Verification items for the finished model (mm, model axes). A direction names the side the tool comes from. Coordinates: 2 decimals unless noted, no trailing zeros. Order: outer loops, then holes, each group sorted by start corner. A loop starts at its lowest first (then second) coordinate and runs counter-clockwise, first axis right, second up. Notation, with made-up numbers: M 24,0.25 L 31,0.25 A27 ccw 31,25.25 Z; hole C -40,-28.75 d1. An arc over 180 degrees is marked long. Return JSON: item names as keys, results as strings. Group by question number.
1. Section check B-B, the plane z = -107. Record the cut outline in (x, y), plus the area to 3 significant figures.
2. Material ranges on line 1 along X through (y, z) = (258, 5); line 2 along Z through (x, y) = (-108, 240), recorded low to high.
3. Mould release check, pull along X, two halves, no side actions. Record for faces 1 (the flat face through (5, 143, -176.332)), 2 (the flat face through (9, 143, -171.332)), 3 (the flat face through (-143.106, 111, -22)), 4 (the flat face through (151.894, 143, 13)): +X half, -X half, draft (parallel to the pull), parting line (faces both ways), or undercut.
4. Section check C-C, the plane z = 100. Record the cut outline in (x, y), plus the area to 3 significant figures.
5. Section check D-D, the plane y = 256. Record the cut outline in (x, z), plus the area to 3 significant figures.
6. Set-up check for faces 5 (the flat face through (-138.106, 111, -23)), 6 (the flat face through (74.3, 290, -171.5)): record each of +Z, -Z, +X, -X, +Y, -Y from which the full face is reachable in a straight line by a thin tool's end or side.
7. Gauge pin test, flat ends, axial feed: pin 1 (2.5 mm diameter, centred on x = 154.39, y = 25, fed in from -Z); pin 2 (5 mm diameter, centred on x = -35.5, y = 87, fed in from +Z); pin 3 (1.2 mm diameter, centred on x = 154.39, z = 73.67, fed in from -Y). Record the tip position at first contact, or that the pin passes through.
8. Section check A-A, the plane z = 18. Record the cut outline in (x, y).
```python
from build123d import *

# Parameters (mm, degrees)
BOSS_EXTRUDE1_DEPTH         = 290
M2_5_TAPPED_HOLE1_D         = 2.05
M2_5_TAPPED_HOLE1_DEPTH     = 7.25
M2_5_TAPPED_HOLE1_TIP       = 0.615882135
CUT_EXTRUDE2_DEPTH          = 41
CUT_EXTRUDE3_DEPTH          = 56
M4_TAPPED_HOLE1_D           = 3.3
M4_TAPPED_HOLE1_CSINK_D     = 4.05
M4_TAPPED_HOLE1_CSINK_ANGLE = 90
M2_5_TAPPED_HOLE2_D         = 2.05
M2_5_TAPPED_HOLE2_DEPTH     = 7.25
M2_5_TAPPED_HOLE2_TIP       = 0.615882135


with BuildPart() as part:
    # Sketch1 → Boss-Extrude1 (new body)
    with BuildSketch(Plane(origin=(0, 0, 0), x_dir=(1, 0, 0), z_dir=(0, 1, 0))):
        with BuildLine():
            Line((-138.105758434, 176.332217748), (151.894241566, 176.332217748))
            ThreePointArc((151.894241566, 176.332217748), (155.429775472, 174.867751654), (156.894241566, 171.332217748))
            Line((156.894241566, 171.332217748), (156.894241566, -123.667782252))
            Line((156.894241566, -123.667782252), (151.894241566, -123.667782252))
            Line((151.894241566, -123.667782252), (151.894241566, 166.332217748))
            ThreePointArc((151.894241566, 166.332217748), (150.429775472, 169.867751654), (146.894241566, 171.332217748))
            Line((146.894241566, 171.332217748), (-133.105758434, 171.332217748))
            ThreePointArc((-133.105758434, 171.332217748), (-136.64129234, 169.867751654), (-138.105758434, 166.332217748))
            Line((-138.105758434, 166.332217748), (-138.105758434, -123.667782252))
            Line((-138.105758434, -123.667782252), (-143.105758434, -123.667782252))
            Line((-143.105758434, -123.667782252), (-143.105758434, 171.332217748))
            ThreePointArc((-143.105758434, 171.332217748), (-141.64129234, 174.867751654), (-138.105758434, 176.332217748))
        make_face()
    extrude(amount=BOSS_EXTRUDE1_DEPTH)

    # M2.5 Tapped Hole1
    with Locations(Plane.XY.offset(123.667782252)):
        with Locations((-140.605758434, 145), (-140.605758434, 265), (-140.605758434, 25), (154.394241566, 145), (154.394241566, 265), (154.394241566, 25)):
            Hole(M2_5_TAPPED_HOLE1_D / 2, depth=M2_5_TAPPED_HOLE1_DEPTH)
            with Locations((0, 0, -(M2_5_TAPPED_HOLE1_DEPTH + M2_5_TAPPED_HOLE1_TIP / 2))):  # 118° drill point
                Cone(0, M2_5_TAPPED_HOLE1_D / 2, M2_5_TAPPED_HOLE1_TIP, mode=Mode.SUBTRACT)

    # Sketch5 → Cut-Extrude2 (cut)
    with BuildSketch(Plane.ZY.offset(143.105758434)):
        with BuildLine():
            Line((-116.332217748, 147.1), (33.667782252, 147.1))
            ThreePointArc((33.667782252, 147.1), (35.767782252, 145), (33.667782252, 142.9))
            Line((33.667782252, 142.9), (-116.332217748, 142.9))
            ThreePointArc((-116.332217748, 142.9), (-118.432217748, 145), (-116.332217748, 147.1))
        make_face()
    extrude(amount=-CUT_EXTRUDE2_DEPTH, mode=Mode.SUBTRACT)

    # Sketch6 → Cut-Extrude3 (cut)
    with BuildSketch(Plane(origin=(156.894241566, 0, 0), x_dir=(0, 0, -1), z_dir=(1, 0, 0))):
        with BuildLine():
            Line((6.018226887, 148.1), (146.332217748, 148.1))
            ThreePointArc((146.332217748, 148.1), (149.432217748, 145), (146.332217748, 141.9))
            Line((146.332217748, 141.9), (6.018226887, 141.9))
            ThreePointArc((6.018226887, 141.9), (2.918226887, 145), (6.018226887, 148.1))
        make_face()
    extrude(amount=-CUT_EXTRUDE3_DEPTH, mode=Mode.SUBTRACT)

    # M4 Tapped Hole1 (through all)
    with Locations(Plane(origin=(156.894241566, 0, 0), x_dir=(0, 0, -1), z_dir=(1, 0, 0))):
        with Locations((-115.667782252, 220), (-115.667782252, 70)):
            CounterSinkHole(M4_TAPPED_HOLE1_D / 2, M4_TAPPED_HOLE1_CSINK_D / 2, counter_sink_angle=M4_TAPPED_HOLE1_CSINK_ANGLE)

    # M2.5 Tapped Hole2
    with Locations(Plane(origin=(0, 0, 0), x_dir=(-1, 0, 0), z_dir=(0, -1, 0))):
        with Locations((-154.394241566, 136.332217748), (-154.394241566, 86.332217748), (-154.394241566, 6.332217748), (-154.394241566, -73.667782252), (-121.894241566, 173.832217748), (-51.894241566, 173.832217748), (38.105758434, 173.832217748), (108.105758434, 173.832217748), (140.605758434, -73.667782252), (140.605758434, 6.332217748), (140.605758434, 86.332217748), (140.605758434, 136.332217748)):
            Hole(M2_5_TAPPED_HOLE2_D / 2, depth=M2_5_TAPPED_HOLE2_DEPTH)
            with Locations((0, 0, -(M2_5_TAPPED_HOLE2_DEPTH + M2_5_TAPPED_HOLE2_TIP / 2))):  # 118° drill point
                Cone(0, M2_5_TAPPED_HOLE2_D / 2, M2_5_TAPPED_HOLE2_TIP, mode=Mode.SUBTRACT)


solid = part.part
```
Answers follow:
{
 "1": {"outline": "M -143.11,0 L -138.11,0 L -138.11,142.9 L -143.11,142.9 Z; M -143.11,147.1 L -138.11,147.1 L -138.11,290 L -143.11,290 Z; M 151.89,0 L 156.89,0 L 156.89,141.9 L 151.89,141.9 Z; M 151.89,148.1 L 156.89,148.1 L 156.89,290 L 151.89,290 Z", "area": "2,850 mm^2"},
 "2": {"line 1": "-143.11 to -138.11, 151.89 to 156.89", "line 2": "-176.33 to -171.33"},
 "3": {"face 1": "draft", "face 2": "undercut", "face 3": "-X half", "face 4": "undercut"},
 "4": {"outline": "M -143.11,0 L -138.11,0 L -138.11,290 L -143.11,290 Z; M 151.89,0 L 156.89,0 L 156.89,290 L 151.89,290 Z", "area": "2,900 mm^2"},
 "5": {"outline": "M -143.11,-171.33 A5 ccw -138.11,-176.33 L 151.89,-176.33 A5 ccw 156.89,-171.33 L 156.89,123.67 L 151.89,123.67 L 151.89,-166.33 A5 cw 146.89,-171.33 L -133.11,-171.33 A5 cw -138.11,-166.33 L -138.11,123.67 L -143.11,123.67 Z", "area": "4,450 mm^2"},
 "6": {"face 5": "+Z, +Y, -Y", "face 6": "+Z, -Z, +X, -X, +Y"},
 "7": {"pin 1": "z = -176.17", "pin 2": "z = -171.33", "pin 3": "y = 7.5"},
 "8": {"outline": "M -143.11,0 L -138.11,0 L -138.11,142.9 L -143.11,142.9 Z; M -143.11,147.1 L -138.11,147.1 L -138.11,290 L -143.11,290 Z; M 151.89,0 L 156.89,0 L 156.89,290 L 151.89,290 Z"}
}
